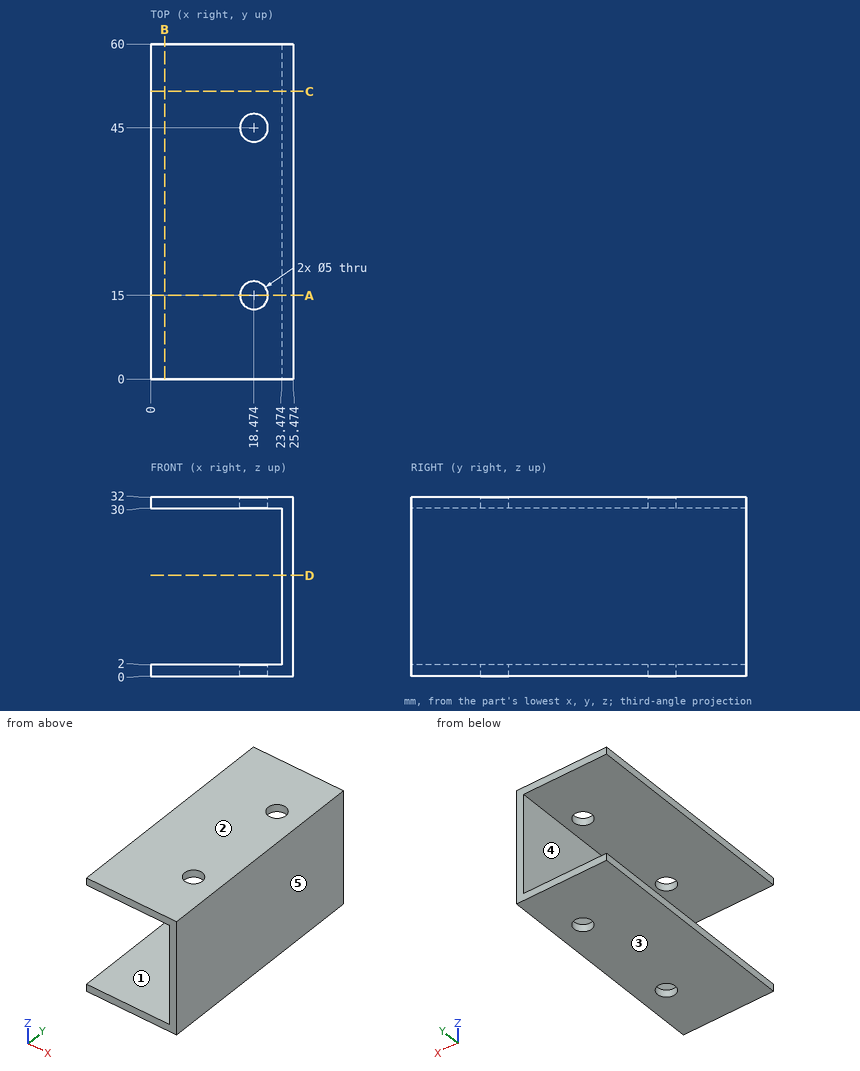
Could you check a few things on this drawing? It's one solid part, dimensions in mm from its lowest x, y, z. A direction names the side the tool comes from. Coordinates: 2 decimals unless noted, no trailing zeros. Write each loop counter-clockwise with the first axis right and the second up, starting at its lowest first coordinate (ties: lowest second). Pieces come first, ordered by that corner, then holes.
Q1. Imagine slicing it at B-B, the plane x = 2.5. List the corners of the cut face in (y, z) for me.
Results found:
outline: (0, 0) - (60, 0) - (60, 2) - (0, 2) - close; (0, 30) - (60, 30) - (60, 32) - (0, 32) - close
Q2. Please list where these lines run through material, in increasing order: L1, parallel to Z at x = 17.5, y = 41.5; L2, parallel to X at y = 30, z = 8.
Results found:
L1: z = 0 to 2, 30 to 32
L2: x = 23.47 to 25.47
Q3. For P1, Ø1, axis at x = 14, z = 3.5, coming from the -Y side; P2, Ø14, axis at y = 33, z = 22.5, coming from the -X side, each with a flat end and sliding along its axis, tell me the tip position at first contact or that it passes through.
Results found:
P1: passes through
P2: stops at x = 23.47
Q4. If we mould it in two halves opening along Z, with no side actions, what happens to the marked faces 1, 2 and 3? For each: +Z half, -Z half, draft (parallel to the pull), parting line (faces both ways), or undercut.
Results found:
face 1: undercut
face 2: +Z half
face 3: -Z half
Q5. Imagine slicing it at C-C, the plane y = 51.5. List the corners of the cut face in (x, z) for me, plus the area to 3 significant figures.
Results found:
outline: (0, 0) - (25.47, 0) - (25.47, 32) - (0, 32) - (0, 30) - (23.47, 30) - (23.47, 2) - (0, 2) - close
area: 158 mm2
Q6. Which directions (+Z, -Z, +X, -X, +Y, -Y) give clear straight access to the entire face, cutting with the end or side of a thin tool? Please do the marked faces 4 and 5.
Results found:
face 4: -X, +Y, -Y
face 5: +Z, -Z, +X, +Y, -Y
Q7. Imagine slicing it at A-A, the plane y = 15. List the corners of the cut face in (x, z) for me, plus the area to 3 significant figures.
Results found:
outline: (0, 0) - (15.97, 0) - (15.97, 2) - (0, 2) - close; (0, 30) - (15.97, 30) - (15.97, 32) - (0, 32) - close; (20.97, 0) - (25.47, 0) - (25.47, 32) - (20.97, 32) - (20.97, 30) - (23.47, 30) - (23.47, 2) - (20.97, 2) - close
area: 138 mm2
Q8. Imagine slicing it at D-D, the plane z = 18. List the corners of the cut face in (x, y) for me.
Results found:
outline: (23.47, 0) - (25.47, 0) - (25.47, 60) - (23.47, 60) - close
